```python
from build123d import *
from build123d.topology import SkipClean

# Parameters (mm, degrees)
SKETCH_1_R          = 90
SKETCH_1_R_2        = 25
SKETCH_1_R_3        = 5.25
EXTRUDE_1_DEPTH     = 15
EXTRUDE_START       = 20
SKETCH_2_R          = 55
SKETCH_2_R_2        = 25
EXTRUDE_2_DEPTH     = 20
SKETCH_3_R          = 45
CUT_EXTRUDE_1_DEPTH = 20
FILLET_1_R          = 3


with BuildPart() as part:
    # 草图1 → 凸台-拉伸1 (new body)
    with BuildSketch(Plane.XY):
        Circle(SKETCH_1_R)
        Circle(SKETCH_1_R_2, mode=Mode.SUBTRACT)
        with Locations((0, 75)):
            Circle(SKETCH_1_R_3, mode=Mode.SUBTRACT)
        with Locations((64.951905284, 37.5)):
            Circle(SKETCH_1_R_3, mode=Mode.SUBTRACT)
        with Locations((64.951905284, -37.5)):
            Circle(SKETCH_1_R_3, mode=Mode.SUBTRACT)
        with Locations((0, -75)):
            Circle(SKETCH_1_R_3, mode=Mode.SUBTRACT)
        with Locations((-64.951905284, -37.5)):
            Circle(SKETCH_1_R_3, mode=Mode.SUBTRACT)
        with Locations((-64.951905284, 37.5)):
            Circle(SKETCH_1_R_3, mode=Mode.SUBTRACT)
    extrude(amount=EXTRUDE_1_DEPTH)

    # 草图2 → 凸台-拉伸2 (add)
    with SkipClean():  # the faces are left unmerged after this step: merging them gives an invalid solid
        with BuildSketch(Plane(origin=(0, 0, 0), x_dir=(-1, 0, 0), z_dir=(0, 0, -1)).offset(EXTRUDE_START)):
            with Locations(Location((0, 0, 0), (0, 0, 180))):
                Circle(SKETCH_2_R)
            Circle(SKETCH_2_R_2, mode=Mode.SUBTRACT)
        extrude(amount=-EXTRUDE_2_DEPTH)

    # 草图3 → 切除-拉伸1 (cut)
    with BuildSketch(Plane.XY.offset(15)):
        Circle(SKETCH_3_R)
    extrude(amount=-CUT_EXTRUDE_1_DEPTH, mode=Mode.SUBTRACT)

    # 圆角1
    fillet_1_edges = [part.edges().sort_by_distance(p)[0] for p in [
        (-90, 0, 0),
        (-55, 0, 0),
        (-55, 0, -20),
    ]]
    fillet(fillet_1_edges, radius=FILLET_1_R)


solid = part.part
```
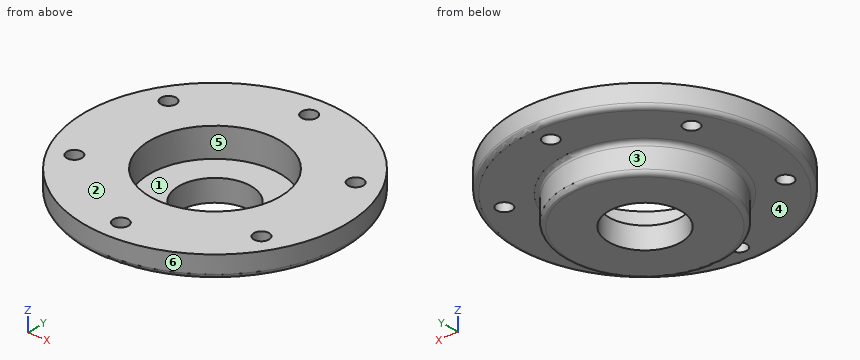
Work out the finished part from the listing and answer in its coordinate system (mm). Face numbers are marked on the shaded views. A direction names the side the tool comes from. Round coordinates to 2 decimals unless told otherwise and drop trailing zeros. Write each loop counter-clockwise with the first axis right and the second up, starting at its lowest first coordinate (ties: lowest second). Pieces come first, ordered by that corner, then holes. Notation, with made-up numbers: (82, 10.25) -> (136, 10.25) arc R18 cw to (136, 35.25) -> close; hole circle Ø2 at (37, 82.5). An arc over 180 degrees is marked (long way). Write each question's results on one line, items separated by ' | '.
1) The part is cut by section B-B (y = 0). Write down the section's boundary in (x, z), and give its area (3 significant figures).
Findings:
outline: (-90, 3) arc R3 ccw to (-87, 0) -> (-58, 0) arc R3 cw to (-55, -3) -> (-55, -17) arc R3 ccw to (-52, -20) -> (-25, -20) -> (-25, -5) -> (-45, -5) -> (-45, 15) -> (-90, 15) -> close; (25, -20) -> (52, -20) arc R3 ccw to (55, -17) -> (55, -3) arc R3 cw to (58, 0) -> (87, 0) arc R3 ccw to (90, 3) -> (90, 15) -> (45, 15) -> (45, -5) -> (25, -5) -> close | area: 2,350 mm²
2) Which of the six approach directions +Z, -Z, +X, -X, +Y, -Y give full straight-line access (tool end or side, diameter ignored) to the marked faces 4, 5 and 6?
Findings:
face 4: -Z | face 5: +Z | face 6: +Z, -Z
3) Flat-ended cylindrical pins translate along their axes: pin 1 (12 mm diameter, centred on x = 25, y = 23.5, fed in from +Z); pin 2 (12 mm diameter, centred on x = 0, y = 75, fed in from -Z); pin 3 (6 mm diameter, centred on x = 4.5, z = 4, fed in from +Y). Find the tip coordinate at first contact, or state that the pin passes through.
Findings:
pin 1: stops at z = -5 | pin 2: stops at z = 0 | pin 3: stops at y = 89.99
4) Consider line 1 along Y through (x, z) = (0, 11); line 2 along Y through (x, z) = (0, -15.5); line 3 along X through (y, z) = (37, 6). Determine where each line is inside the solid, lowest interval first. Write a range as [from, to].
Findings:
line 1: y = [-90, -80.25], [-69.75, -45], [45, 69.75], [80.25, 90] | line 2: y = [-55, -25], [25, 55] | line 3: x = [-82.04, -70.18], [-59.73, -25.61], [25.61, 59.73], [70.18, 82.04]
5) For a pull along X with two mould halves and no side action, classify the marked faces 1, 2 and 3 as +X half, -X half, draft (parallel to the pull), parting line (faces both ways), or undercut.
Findings:
face 1: undercut | face 2: draft | face 3: parting line
6) The part is cut by section C-C (z = 7). Write down the section's boundary in (x, y), and give its area (3 significant figures).
Findings:
outline: circle Ø180 at (0, 0); hole circle Ø10.5 at (-64.95, -37.5); hole circle Ø10.5 at (-64.95, 37.5); hole circle Ø90 at (0, 0); hole circle Ø10.5 at (0, -75); hole circle Ø10.5 at (0, 75); hole circle Ø10.5 at (64.95, -37.5); hole circle Ø10.5 at (64.95, 37.5) | area: 18,600 mm²
7) The part is cut by section A-A (x = 0). State how many separate pieces and enclosed holes the cut face has, and give its area (3 significant figures).
Findings:
separate pieces: 4 | enclosed holes: 0 | area: 2,030 mm²
8) The part is cut by section D-D (z = -9). Write down the section's boundary in (x, y), and give its area (3 significant figures).
Findings:
outline: circle Ø110 at (0, 0); hole circle Ø50 at (0, 0) | area: 7,540 mm²
